from build123d import *

# Parameters (mm, degrees)
BOSS_EXTRUDE1_DEPTH = 1.5
SKETCH2_W           = 1200
SKETCH2_H           = 1.5
BOSS_EXTRUDE2_DEPTH = 5


with BuildPart() as part:
    # Sketch1 → Boss-Extrude1 (new body)
    with BuildSketch(Plane.XY):
        Polygon((40, 0), (1240, 0), (1240, 40), (1280, 40), (1280, 390), (1240, 390), (1240, 430), (40, 430), (40, 390), (0, 390), (0, 40), (40, 40), align=None)
    extrude(amount=BOSS_EXTRUDE1_DEPTH)

    # Sketch2 → Boss-Extrude2 (add)
    with BuildSketch(Plane.XY.offset(1.5)):
        with Locations((640, 429.25)):
            Rectangle(SKETCH2_W, SKETCH2_H)
        with Locations((640, 0.75)):
            Rectangle(SKETCH2_W, SKETCH2_H)
    extrude(amount=BOSS_EXTRUDE2_DEPTH)


solid = part.part
Check sheet for the modelled part. Datum: model origin and axes. Units: mm. Round coordinates to 2 decimals unless told otherwise and drop trailing zeros. Loops run counter-clockwise (first coordinate to the right, second up) from the corner with the lowest first, then second, coordinate; pieces in that order, holes last. Notation, with made-up numbers: (73, 76) -> (130, 76) arc R11 ccw to (130, 86) -> close; hole circle Ø2 at (52.25, -17.5). An arc over 180 degrees is marked (long way). Put each result on its own line as item: value. Start each with the question number.
1. Section check B-B (x = 116.5). Enter the section's corners in (y, z).
2. Scan lines: probe 1 along Y at (x, z) = (426, 4.5); probe 2 along Z at (x, y) = (1152, 185.5). Record each from-to range of solid material in increasing order.
3. Gauge pin test, flat ends, axial feed: pin 1 (1.6 mm diameter, centred on x = 1264.5, z = 0.5, fed in from -Y); pin 2 (1.6 mm diameter, centred on x = 17.5, z = 0.5, fed in from +Y); pin 3 (3 mm diameter, centred on y = 419.5, z = 4.5, fed in from -X); pin 4 (1 mm diameter, centred on x = 619.5, y = 361.5, fed in from +Z). Record the tip position at first contact, or that the pin passes through.
4. Draft check along Y on faces 1 (the face through (631, 218, 1.5)), 2 (the face through (631, 218, 0)). Enter one of: +Y half, -Y half, draft (parallel to the pull), parting line (faces both ways), or undercut.
5. Section check A-A (z = 2.5). Enter the section's corners in (x, y).
6. Section check C-C (y = 376). Enter the section's corners in (x, z).
Findings:
1. outline: (0, 0) -> (430, 0) -> (430, 6.5) -> (428.5, 6.5) -> (428.5, 1.5) -> (1.5, 1.5) -> (1.5, 6.5) -> (0, 6.5) -> close
2. probe 1: y = 0 to 1.5, 428.5 to 430
2. probe 2: z = 0 to 1.5
3. pin 1: stops at y = 40
3. pin 2: stops at y = 390
3. pin 3: passes through
3. pin 4: stops at z = 1.5
4. face 1: undercut
4. face 2: draft
5. outline: (40, 0) -> (1240, 0) -> (1240, 1.5) -> (40, 1.5) -> close; (40, 428.5) -> (1240, 428.5) -> (1240, 430) -> (40, 430) -> close
6. outline: (0, 0) -> (1280, 0) -> (1280, 1.5) -> (0, 1.5) -> close
